Source: CAD feature listing. Evaluate the final solid. Frame: model axes, mm. Give positions to 0.01 mm unless a question says otherwise; leave off trailing zeros. Order: outer loops, then holes, each group sorted by start corner. A loop starts at its lowest first (then second) coordinate and runs counter-clockwise, first axis right, second up.
```python
from build123d import *

# Parameters (mm, degrees)
SKETCH1_R             = 10
BOSS_EXTRUDE1_DEPTH   = 400
M6_TAPPED_HOLE1_D     = 5
M6_TAPPED_HOLE1_DEPTH = 15
M6_TAPPED_HOLE1_TIP   = 1.502151548
M6_TAPPED_HOLE2_D     = 5
M6_TAPPED_HOLE2_DEPTH = 15
M6_TAPPED_HOLE2_TIP   = 1.502151548


with BuildPart() as part:
    # Sketch1 → Boss-Extrude1 (new body)
    with BuildSketch(Plane.XY):
        Circle(SKETCH1_R)
    extrude(amount=BOSS_EXTRUDE1_DEPTH)

    # M6 Tapped Hole1
    with Locations(Plane.XY.offset(400)):
        with Locations((0, 0)):
            Hole(M6_TAPPED_HOLE1_D / 2, depth=M6_TAPPED_HOLE1_DEPTH)
            with Locations((0, 0, -(M6_TAPPED_HOLE1_DEPTH + M6_TAPPED_HOLE1_TIP / 2))):  # 118° drill point
                Cone(0, M6_TAPPED_HOLE1_D / 2, M6_TAPPED_HOLE1_TIP, mode=Mode.SUBTRACT)

    # M6 Tapped Hole2
    with Locations(Plane(origin=(0, 0, 0), x_dir=(-1, 0, 0), z_dir=(0, 0, -1))):
        with Locations((0, 0)):
            Hole(M6_TAPPED_HOLE2_D / 2, depth=M6_TAPPED_HOLE2_DEPTH)
            with Locations((0, 0, -(M6_TAPPED_HOLE2_DEPTH + M6_TAPPED_HOLE2_TIP / 2))):  # 118° drill point
                Cone(0, M6_TAPPED_HOLE2_D / 2, M6_TAPPED_HOLE2_TIP, mode=Mode.SUBTRACT)


solid = part.part
```
1) Pin query (flat end, axial travel): pin 1 (1 mm diameter, centred on x = 2, z = 266.5, fed in from +Y); pin 2 (3 mm diameter, centred on x = 2, z = 109, fed in from +Y); pin 3 (1 mm diameter, centred on y = -1, z = 55, fed in from +X). Return the tip coordinate at first contact, or that it passes through.
Report:
pin 1: stops at y = 9.89
pin 2: stops at y = 9.99
pin 3: stops at x = 9.99
2) Section query B-B, the plane y = -6. Return the cut outline in (x, z).
Report:
outline: (-8, 0) - (8, 0) - (8, 400) - (-8, 400) - close
3) Material intervals for L1, parallel to Y at x = 0, z = 396.25; L2, parallel to Y at x = 2.5, z = 64; L3, parallel to Y at x = -4.75, z = 338, sorted ascending.
Report:
L1: y = -10 to -2.5, 2.5 to 10
L2: y = -9.68 to 9.68
L3: y = -8.8 to 8.8
4) Section query A-A, the plane z = 198. Return the cut outline in (x, y).
Report:
outline: circle Ø20 at (0, 0)
